Source: CAD feature listing. Evaluate the final solid. Frame: model axes, mm. Give positions to 0.01 mm unless a question says otherwise; leave off trailing zeros. Order: outer loops, then holes, each group sorted by start corner. A loop starts at its lowest first (then second) coordinate and runs counter-clockwise, first axis right, second up. Notation, with made-up numbers: (-37, 46.5) - (13, 46.5) arc R13 cw to (13, 55.5) - close; hole circle Ø4 at (71.25, 81). An arc over 180 degrees is marked (long way). Use CSV: the item, a comma, the result in double quotes.
```python
from build123d import *

# Parameters (mm, degrees)
SKETCH2_R           = 15
BOSS_EXTRUDE1_DEPTH = 15


with BuildPart() as part:
    # Sketch2 → Boss-Extrude1 (new body)
    with BuildSketch(Plane(origin=(0, 0, 0), x_dir=(1, 0, 0), z_dir=(0, 1, 0))):
        with BuildLine():
            Line((25, 0), (25, -31.912942224))
            Line((25, -31.912942224), (-25, -31.912942224))
            Line((-25, -31.912942224), (-25, 0))
            ThreePointArc((-25, 0), (0, 25), (25, 0))
        make_face()
        with Locations(Location((0, 0, 0), (0, 0, 270))):
            Circle(SKETCH2_R, mode=Mode.SUBTRACT)
    boss_extrude1 = extrude(amount=BOSS_EXTRUDE1_DEPTH)

    # Sketch4 → Revolve1 (revolve)
    with BuildSketch(Plane(origin=(0, -12, 0), x_dir=(-1, 0, 0), z_dir=(0, -1, 0))):
        Polygon((0, -31.912942224), (29.933248422, -31.912942224), (29.933248422, -39.086469166), (22.382657632, -39.086469166), (22.382657632, -44.842453341), (29.933248422, -44.842453341), (22, -389.086469166), (14, -389.086469166), (14, -39.086469166), (0, -39.086469166), align=None)
    revolve(axis=Axis((0, -12, 31.912942224), (0, 0, 1)))

    # Mirror5: Boss-Extrude1 across plane
    add(boss_extrude1.mirror(Plane(origin=(0, -12, 0), x_dir=(0, 0, 1), z_dir=(0, -1, 0))))


solid = part.part
```
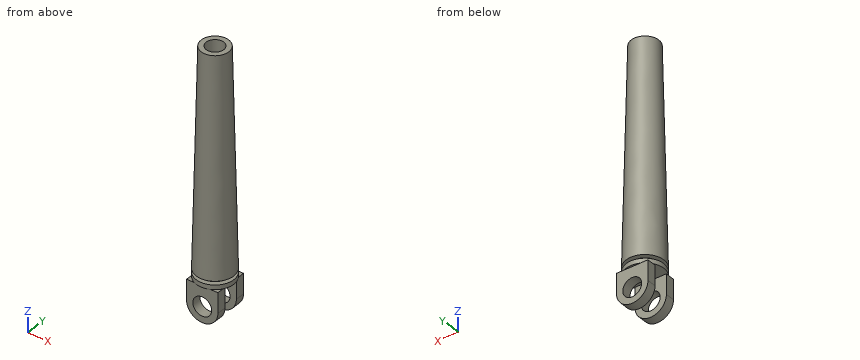
Item 1: Section C-C on z = 239. Return the cut outline in (x, y).
Filled in:
outline,"circle Ø50.92 at (0, -12); hole circle Ø28 at (0, -12)"
Item 2: Section B-B on y = -12. Return the cut outline in (x, z), then the cut area to 3 significant figures.
Filled in:
outline,"(-29.93, 31.91) - (29.93, 31.91) - (29.93, 39.09) - (22.38, 39.09) - (22.38, 44.84) - (29.93, 44.84) - (22, 389.09) - (14, 389.09) - (14, 39.09) - (-14, 39.09) - (-14, 389.09) - (-22, 389.09) - (-29.93, 44.84) - (-22.38, 44.84) - (-22.38, 39.09) - (-29.93, 39.09) - close"
area,"8,760 mm2"
Item 3: First-contact query: pin 1 (25 mm diameter, centred on x = 7, z = 4.5, fed in from +Y); pin 2 (1.5 mm diameter, centred on x = -3.5, y = -8, fed in from +Z); pin 3 (10 mm diameter, centred on x = 16.5, z = 167.5, fed in from -Y). Flat tips, straight axial feed; report the tip coordinate or a pass-through.
Filled in:
pin 1,"stops at y = 15"
pin 2,"stops at z = 39.09"
pin 3,"stops at y = -36.55"
Item 4: Section D-D on z = 169. Return the cut outline in (x, y).
Filled in:
outline,"circle Ø54.14 at (0, -12); hole circle Ø28 at (0, -12)"
Item 5: Section A-A on x = 0. Count the separate pieces of the cut face and the enclosed holes in it, then the cut area to 3 significant figures.
Filled in:
separate pieces,"3"
enclosed holes,"0"
area,"9,570 mm2"
Item 6: Material intervals for line 1 (X direction, y = 6, z = 0); line 2 (Y direction, x = 8, z = 361); line 3 (Y direction, x = 4, z = 316), sorted ascending. Write a range as from..to.
Filled in:
line 1,"x = -25..-15, 15..25"
line 2,"y = -33.19..-23.49, -0.51..9.19"
line 3,"y = -35.34..-25.42, 1.42..11.34"
